from build123d import *

# Parameters (mm, degrees)
SKETCH1_W           = 250
SKETCH1_H           = 200
BOSS_EXTRUDE1_DEPTH = 10
M6_TAPPED_HOLE1_D   = 5


with BuildPart() as part:
    # Sketch1 → Boss-Extrude1 (new body)
    with BuildSketch(Plane.XY):
        Rectangle(SKETCH1_W, SKETCH1_H)
    extrude(amount=BOSS_EXTRUDE1_DEPTH)

    # M6 Tapped Hole1 (through all)
    with Locations(Plane.XY.offset(10)):
        with Locations((-85.5, 62), (-28.5, 62), (85.5, 62), (28.5, 62), (28.5, -62), (85.5, -62), (-28.5, -62), (-85.5, -62)):
            Hole(M6_TAPPED_HOLE1_D / 2)


solid = part.part
Could you check a few things on this model? Use its own coordinates, in mm. Give positions to 0.01 mm unless a question says otherwise; leave off trailing zeros. Answer as CSV lines item,"result". Start each with the question number.
(1) I'm going to push flat-ended pins straight in: pin 1 Ø6.5 at (x, y) = (-85.5, 62) entering from -Z; pin 2 Ø4 at (x, y) = (28.5, 62) entering from -Z. Where does each tip first touch, or does it pass through?
(2) We'd pull the mould along X, two halves only. Please class faces 1 (the cylindrical face through (-83, 62, 5)), 2 (the flat face through (-2, -100, 5)), 3 (the flat face through (125, -1, 5)): released by +X, released by -X, zero draft, split by the parting line, or undercut.
(3) I need wall thicknesses on probe 1 along Y at (x, z) = (-85.5, 4). Which ranges of the line are inside material? Lowest first, please.
Computed:
1,pin 1,"stops at z = 0"
1,pin 2,"passes through"
2,face 1,"undercut"
2,face 2,"zero draft"
2,face 3,"released by +X"
3,probe 1,"y = -100 to -64.5, -59.5 to 59.5, 64.5 to 100"
